For this review, use the dimensioned drawing (mm, ordinates from the lowest corner) and the shaded views. A direction names the side the tool comes from. Give positions to 0.01 mm unless a question says otherwise; leave off trailing zeros. Write each loop counter-clockwise with the first axis right and the second up, starting at its lowest first coordinate (ties: lowest second). Pieces come first, ordered by that corner, then holes.
1) Draft analysis for pull direction Y (two halves, no side actions). For the marked faces 1, 2 and 3, state which applies: pulls with the +Y half, pulls with the -Y half, needs draft (parallel to the pull), parting line crosses it, or undercut.
2) We need section D-D on z = 3.75. Give the boundary of the cut face in (x, y), and give its area (3 significant figures).
3) For P1, Ø1, axis at x = 4.5, z = 6, coming from the +Y side; P2, Ø2, axis at x = 6, z = 13.5, coming from the +Y side, all flat-tipped, find the tip position at first contact; note any pin that passes through.
4) We need section C-C on x = 6. Give the boundary of the cut face in (y, z).
5) Wall thickness on line 1 along Y through (x, z) = (4.75, 7.5); line 2 along Y through (x, z) = (1.65, 7.5): over which ranges is each line inside the solid? List them lowest first.
6) We need section A-A on y = 7.5. Give the boundary of the cut face in (x, z).
7) Machinability: for the marked faces 4 and 5, which of the approach directions +Z, -Z, +X, -X, +Y, -Y give a long, thin tool a straight path to every point of the face, cutting with its end or side? Answer none if there is none.
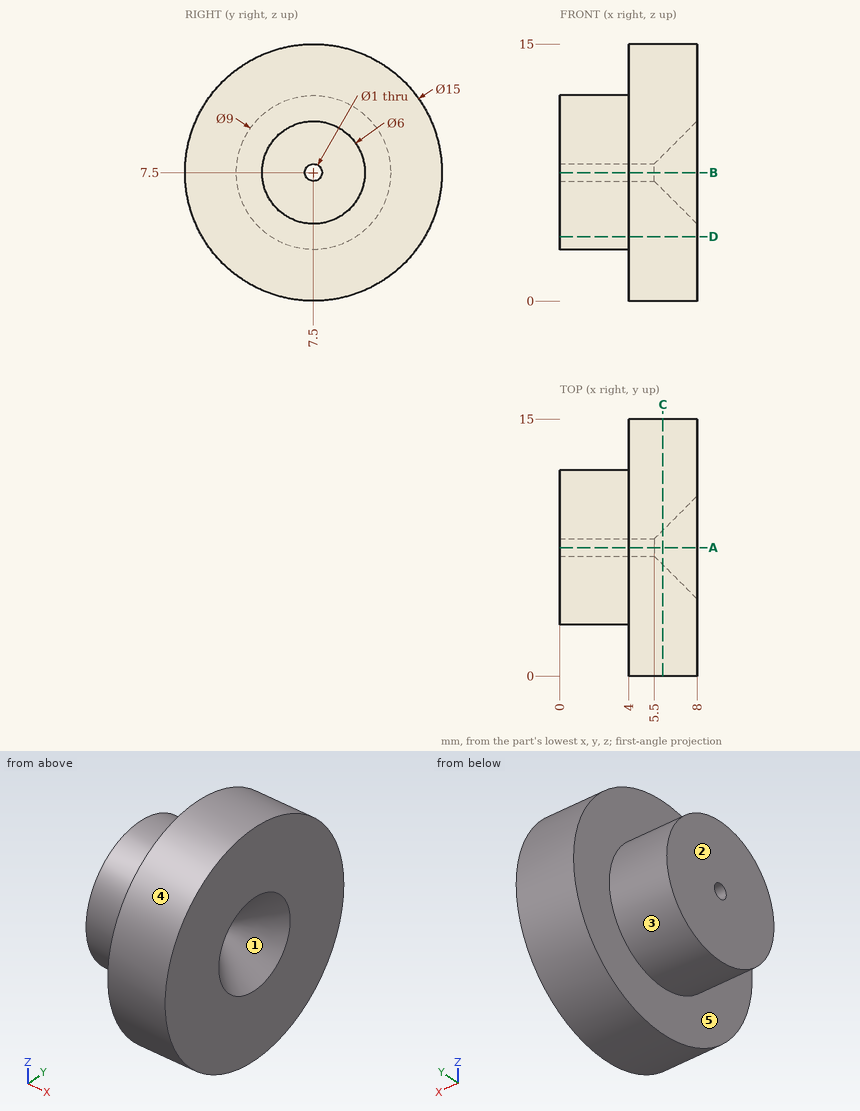
Results list:
1. face 1: undercut
1. face 2: needs draft
1. face 3: parting line crosses it
2. outline: (0, 5.01) - (4, 5.01) - (4, 1) - (8, 1) - (8, 14) - (4, 14) - (4, 9.99) - (0, 9.99) - close
2. area: 71.9 mm2
3. P1: stops at y = 14.93
3. P2: stops at y = 13.09
4. outline: circle Ø15 at (7.5, 7.5); hole circle Ø2 at (7.5, 7.5)
5. line 1: y = 0 to 7, 8 to 15
5. line 2: y = 3 to 7, 8 to 12
6. outline: (0, 3) - (4, 3) - (4, 0) - (8, 0) - (8, 4.5) - (5.5, 7) - (0, 7) - close; (0, 8) - (5.5, 8) - (8, 10.5) - (8, 15) - (4, 15) - (4, 12) - (0, 12) - close
7. face 4: +X, -X
7. face 5: -X
